Design review of the part built by this model. Coordinates are the model's own, in mm. Face numbers are marked on the shaded views. A direction names the side the tool comes from. Round coordinates to 2 decimals unless told otherwise and drop trailing zeros. Return JSON: item names as keys, results as strings. Group by question number.
(1) Clearance check with flat-ended pins moving along their axes: pin 1 (12 mm diameter, centred on x = -2, z = -12.5, fed in from +Y); pin 2 (15 mm diameter, centred on y = 82.5, z = -93.5, fed in from -X); pin 3 (12.5 mm diameter, centred on y = 237, z = 50.5, fed in from +X); pin 4 (4 mm diameter, centred on x = -46.5, z = -56.5, fed in from -Y). State where each tip first meets the part, or that it passes through.
(2) Wall thickness on L1, parallel to X at y = 58.5, z = 8; L2, parallel to Y at x = -57, z = -26.5; L3, parallel to X at y = 46.5, z = -81.5: over which ranges is each line inside the solid? List them lowest first. Write a range as [from, to].
(3) The part is to be moulded in two halves that separate along Z. For the marked faces 4, 5, 6 and 7, say which applies: pulls with the +Z half, pulls with the -Z half, needs draft (parallel to the pull), parting line crosses it, or undercut.
(4) For the marked faces 1, 2 and 3, list the 3-axis set-ups (+Z, -Z, +X, -X, +Y, -Y) from which the entire face can be reached by the end or side of a thin tool; tool diameter is ignored.
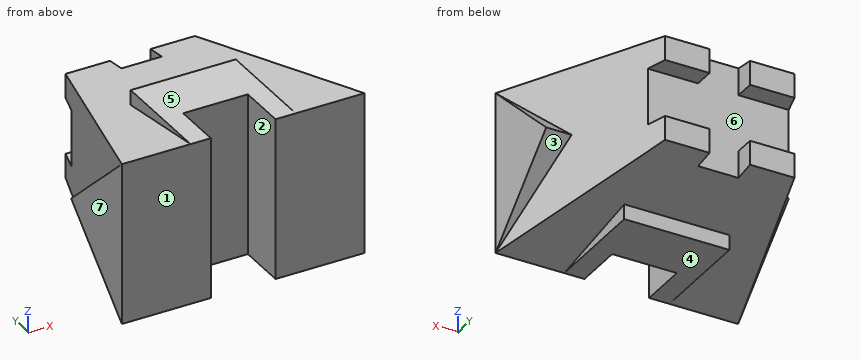
from build123d import *

# Parameters (mm, degrees)
GATE_BLOCK_PROFILE_130X130_W   = 130
GATE_BLOCK_PROFILE_130X130_H   = 130
GATE_BLOCK_DEPTH               = 100
SIDE_BUTTRESS_DEPTH            = 150
DOORWAY_CUT_DEPTH              = 305.179223648
DOORWAY_CUT_DEPTH_BACK         = 305.179223648
DOORWAY_PROFILE_60X80_W        = 80
DOORWAY_PROFILE_60X80_H        = 60
CRENELLATION_CUT_25_DEEP_DEPTH = 25


with BuildPart() as part:
    # Top Profile 160x130 → Pyramidal Body Loft section 0
    with BuildSketch(Plane(origin=(0, 245, 0), x_dir=(1, 0, 0), z_dir=(0, 1, 0))):
        with BuildLine():
            Line((-80, -65), (80, -65))
            Line((80, -65), (80, 65))
            Line((80, 65), (-80, 65))
            Line((-80, 65), (-80, -65))
        make_face()
    # Base Profile 300x200 → Pyramidal Body Loft section 1
    with BuildSketch(Plane(origin=(0, 0, 0), x_dir=(1, 0, 0), z_dir=(0, 1, 0))):
        with BuildLine():
            Line((-150, -100), (150, -100))
            Line((150, -100), (150, 100))
            Line((150, 100), (-150, 100))
            Line((-150, 100), (-150, -100))
        make_face()
    loft()

    # Gate Block Profile 130x130 → Gate Block (add, symmetric)
    with BuildSketch(Plane.XY):
        with Locations((0, 65)):
            Rectangle(GATE_BLOCK_PROFILE_130X130_W, GATE_BLOCK_PROFILE_130X130_H)
    extrude(amount=GATE_BLOCK_DEPTH, both=True)

    # Side Buttress Profile → Side Buttress (add, symmetric)
    with BuildSketch(Plane(origin=(0, 0, 0), x_dir=(0, 0, -1), z_dir=(1, 0, 0))):
        Polygon((-100, 0), (0, 110), (100, 0), align=None)
    extrude(amount=SIDE_BUTTRESS_DEPTH, both=True)

    # Doorway Profile 60x80 → Doorway Cut (cut, two sides: drawn at the far end of the back side and taken through both)
    with BuildSketch(Plane.XY.offset(-DOORWAY_CUT_DEPTH_BACK)):
        with Locations((0, 30)):
            Rectangle(DOORWAY_PROFILE_60X80_W, DOORWAY_PROFILE_60X80_H)
    extrude(amount=DOORWAY_CUT_DEPTH + DOORWAY_CUT_DEPTH_BACK, mode=Mode.SUBTRACT)

    # Crenellation Profile → Crenellation Cut 25 Deep (cut)
    with BuildSketch(Plane(origin=(0, 245, 0), x_dir=(1, 0, 0), z_dir=(0, 1, 0))):
        Polygon((-25, 65), (-25, 35), (-80, 35), (-93.798877222, 35), (-93.798877222, -35), (-80, -35), (-25, -35), (-25, -65), (-25, -87.972860003), (25, -87.972860003), (25, -65), (25, -35), (80, -35), (94.18727837, -35), (94.18727837, 35), (80, 35), (25, 35), (25, 65), (25, 74.605387162), (-25, 74.605387162), align=None)
    extrude(amount=-CRENELLATION_CUT_25_DEEP_DEPTH, mode=Mode.SUBTRACT)


solid = part.part
Solutions:
{
 "1": {"pin 1": "y = 220", "pin 2": "x = -128.16", "pin 3": "x = 84.07", "pin 4": "y = 0"},
 "2": {"L1": "[-150, -40], [40, 150]", "L2": "[0, 220]", "L3": "[-136.71, -40], [40, 136.71]"},
 "3": {"face 4": "pulls with the -Z half", "face 5": "pulls with the +Z half", "face 6": "undercut", "face 7": "needs draft"},
 "4": {"face 1": "+Z, -Z, +X, -X, -Y", "face 2": "+Z, -Z, -Y", "face 3": "-Z, +X, +Y"}
}
